```python
from build123d import *

# Parameters (mm, degrees)
CUT_EXTRUDE_1_DEPTH      = 88
CUT_EXTRUDE_1_DEPTH_BACK = 88
SKETCH_2_R               = 105
CUT_EXTRUDE_2_DEPTH      = 88
CUT_EXTRUDE_2_DEPTH_BACK = 88
SKETCH_3_R               = 5.5
CUT_EXTRUDE_3_DEPTH      = 88
CUT_EXTRUDE_3_DEPTH_BACK = 88
SKETCH_5_R               = 5.5
CUT_EXTRUDE_4_DEPTH      = 88
CUT_EXTRUDE_4_DEPTH_BACK = 88
SKETCH_6_R               = 5.5
CUT_EXTRUDE_5_DEPTH      = 88
CUT_EXTRUDE_5_DEPTH_BACK = 88
SKETCH_7_R               = 5.5
CUT_EXTRUDE_6_DEPTH      = 88
CUT_EXTRUDE_6_DEPTH_BACK = 88
SKETCH_8_R               = 5.5
CUT_EXTRUDE_7_DEPTH      = 88
CUT_EXTRUDE_7_DEPTH_BACK = 88
SKETCH_9_R               = 5.5
CUT_EXTRUDE_8_DEPTH      = 88
CUT_EXTRUDE_8_DEPTH_BACK = 88
SKETCH_10_R              = 5.5
CUT_EXTRUDE_9_DEPTH      = 88
CUT_EXTRUDE_9_DEPTH_BACK = 88
SKETCH_11_R              = 5.5


with BuildPart() as part:
    # 草图1 → 旋转1 (revolve)
    with BuildSketch(Plane.XY, mode=Mode.PRIVATE) as revolve_1_sk:
        Polygon((0, 37.5), (0, 25), (2, 23), (86, 23), (88, 25), (88, 55), (72, 55), (72, 37.5), align=None)
    revolve(revolve_1_sk.sketch.rotate(Axis((88, 0, 0), (-1, 0, 0)), 270), axis=Axis((88, 0, 0), (-1, 0, 0)))

    # 草图2 → 切除-拉伸1 (cut, two sides: drawn at the far end of the back side and taken through both)
    with BuildSketch(Plane(origin=(0, 0, 0), x_dir=(0, 0, -1), z_dir=(1, 0, 0)).offset(-CUT_EXTRUDE_1_DEPTH_BACK)):
        Circle(SKETCH_2_R)
        with BuildLine():
            Line((-42.5, 82.720916339), (-42.5, -82.720916339))
            ThreePointArc((-42.5, -82.720916339), (0, -93), (42.5, -82.720916339))
            Line((42.5, -82.720916339), (42.5, 82.720916339))
            ThreePointArc((42.5, 82.720916339), (0, 93), (-42.5, 82.720916339))
        make_face(mode=Mode.SUBTRACT)
    extrude(amount=CUT_EXTRUDE_1_DEPTH + CUT_EXTRUDE_1_DEPTH_BACK, mode=Mode.SUBTRACT)

    # 草图3 → 切除-拉伸2 (cut, two sides: drawn at the far end of the back side and taken through both)
    with BuildSketch(Plane(origin=(0, 0, 0), x_dir=(0, 0, -1), z_dir=(1, 0, 0)).offset(-CUT_EXTRUDE_2_DEPTH_BACK)):
        with Locations((-32.880465325, 32.880465325)):
            Circle(SKETCH_3_R)
    extrude(amount=CUT_EXTRUDE_2_DEPTH + CUT_EXTRUDE_2_DEPTH_BACK, mode=Mode.SUBTRACT)

    # 草图5 → 切除-拉伸3 (cut, two sides: drawn at the far end of the back side and taken through both)
    with BuildSketch(Plane(origin=(0, 0, 0), x_dir=(0, 0, -1), z_dir=(1, 0, 0)).offset(-CUT_EXTRUDE_3_DEPTH_BACK)):
        with Locations((-12.035085597, 44.915550922)):
            Circle(SKETCH_5_R)
    extrude(amount=CUT_EXTRUDE_3_DEPTH + CUT_EXTRUDE_3_DEPTH_BACK, mode=Mode.SUBTRACT)

    # 草图6 → 切除-拉伸4 (cut, two sides: drawn at the far end of the back side and taken through both)
    with BuildSketch(Plane(origin=(0, 0, 0), x_dir=(0, 0, -1), z_dir=(1, 0, 0)).offset(-CUT_EXTRUDE_4_DEPTH_BACK)):
        with Locations((12.035085597, 44.915550922)):
            Circle(SKETCH_6_R)
    extrude(amount=CUT_EXTRUDE_4_DEPTH + CUT_EXTRUDE_4_DEPTH_BACK, mode=Mode.SUBTRACT)

    # 草图7 → 切除-拉伸5 (cut, two sides: drawn at the far end of the back side and taken through both)
    with BuildSketch(Plane(origin=(0, 0, 0), x_dir=(0, 0, -1), z_dir=(1, 0, 0)).offset(-CUT_EXTRUDE_5_DEPTH_BACK)):
        with Locations((32.880465325, 32.880465325)):
            Circle(SKETCH_7_R)
    extrude(amount=CUT_EXTRUDE_5_DEPTH + CUT_EXTRUDE_5_DEPTH_BACK, mode=Mode.SUBTRACT)

    # 草图8 → 切除-拉伸6 (cut, two sides: drawn at the far end of the back side and taken through both)
    with BuildSketch(Plane(origin=(0, 0, 0), x_dir=(0, 0, -1), z_dir=(1, 0, 0)).offset(-CUT_EXTRUDE_6_DEPTH_BACK)):
        with Locations((32.880465325, -32.880465325)):
            Circle(SKETCH_8_R)
    extrude(amount=CUT_EXTRUDE_6_DEPTH + CUT_EXTRUDE_6_DEPTH_BACK, mode=Mode.SUBTRACT)

    # 草图9 → 切除-拉伸7 (cut, two sides: drawn at the far end of the back side and taken through both)
    with BuildSketch(Plane(origin=(0, 0, 0), x_dir=(0, 0, -1), z_dir=(1, 0, 0)).offset(-CUT_EXTRUDE_7_DEPTH_BACK)):
        with Locations((12.035085597, -44.915550922)):
            Circle(SKETCH_9_R)
    extrude(amount=CUT_EXTRUDE_7_DEPTH + CUT_EXTRUDE_7_DEPTH_BACK, mode=Mode.SUBTRACT)

    # 草图10 → 切除-拉伸8 (cut, two sides: drawn at the far end of the back side and taken through both)
    with BuildSketch(Plane(origin=(0, 0, 0), x_dir=(0, 0, -1), z_dir=(1, 0, 0)).offset(-CUT_EXTRUDE_8_DEPTH_BACK)):
        with Locations((-12.035085597, -44.915550922)):
            Circle(SKETCH_10_R)
    extrude(amount=CUT_EXTRUDE_8_DEPTH + CUT_EXTRUDE_8_DEPTH_BACK, mode=Mode.SUBTRACT)

    # 草图11 → 切除-拉伸9 (cut, two sides: drawn at the far end of the back side and taken through both)
    with BuildSketch(Plane(origin=(0, 0, 0), x_dir=(0, 0, -1), z_dir=(1, 0, 0)).offset(-CUT_EXTRUDE_9_DEPTH_BACK)):
        with Locations((-32.880465325, -32.880465325)):
            Circle(SKETCH_11_R)
    extrude(amount=CUT_EXTRUDE_9_DEPTH + CUT_EXTRUDE_9_DEPTH_BACK, mode=Mode.SUBTRACT)

    # 草图12 → 切除-旋转1 (revolve, cut)
    with BuildSketch(Plane(origin=(80, 0, 0), x_dir=(0, 0, -1), z_dir=(1, 0, 0)), mode=Mode.PRIVATE) as cut_revolve_1_sk:
        Polygon((7.5, 12.990381057), (4.901923789, 14.490381057), (16.901923789, 35.274990748), (16.621764571, 35.436740748), (24.283514571, 48.707281022), (24.035898385, 49.631397208), (27.5, 47.631397208), align=None)
    revolve(cut_revolve_1_sk.sketch.rotate(Axis((80, 47.631397208, -27.5), (0, -0.8660254037844387, 0.49999999999999983)), 180), axis=Axis((80, 47.631397208, -27.5), (0, -0.8660254037844387, 0.49999999999999983)), mode=Mode.SUBTRACT)


solid = part.part
```
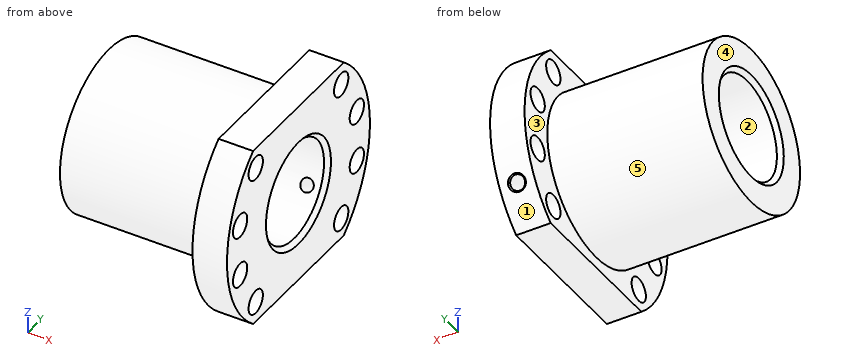
Work out the finished part from the listing and answer in its coordinate system (mm). Face numbers are marked on the shaded views. A direction names the side the tool comes from. Give positions to 0.01 mm unless a question says otherwise; leave off trailing zeros. Order: outer loops, then holes, each group sorted by start corner. A loop starts at its lowest first (then second) coordinate and runs counter-clockwise, first axis right, second up. Notation, with made-up numbers: (6.5, 54) -> (61.5, 54) arc R17 cw to (61.5, 60) -> close; hole circle Ø11 at (63, 11). An arc over 180 degrees is marked (long way). Answer as CSV lines item,"result". Start each with the question number.
(1) Consider line 1 along Z through (x, y) = (81, -32.5); line 2 along Y through (x, z) = (67.5, 0); line 3 along Y through (x, z) = (73, 35.5). Determine where each line is inside the solid, lowest interval first.
(2) For a pull along Y with two mould halves and no side action, classify the marked faces 1, 2 and 3 as released by +Y, released by -Y, zero draft, split by the parting line, or undercut.
(3) Section A-A, the plane z = 0 is taken. Write down the section's boundary in (x, y).
(4) Section B-B, the plane y = 0 is taken. Write down the section's boundary in (x, z), plus the area to 3 significant figures.
(5) Section D-D, the plane x = 53 is taken. Write down the section's boundary in (y, z).
(6) Which of the six approach directions +Z, -Z, +X, -X, +Y, -Y give full straight-line access (tool end or side, diameter ignored) to the marked faces 4 and 5?
(7) Each of these flat-tipped pins is pushed along its axis until it touches: pin 1 Ø12.5 at (y, z) = (32.88, -32.88) entering from -X; pin 2 Ø1 at (x, y) = (49, 13) entering from +Z; pin 3 Ø2 at (x, z) = (68, -30) entering from +Y (3 decimals). Where does it stop, or does it pass through?
(8) Section C-C, the plane y = -29 is taken. Write down the section's boundary in (x, z), plus the area to 3 significant figures.
Entries:
1,line 1,"-42.5 to -38.37, -27.39 to 27.39, 38.37 to 42.5"
1,line 2,"-37.5 to -23, 23 to 37.5"
1,line 3,"-42.01 to -37.72, -28.04 to 28.04, 37.72 to 42.01"
2,face 1,"released by +Y"
2,face 2,"undercut"
2,face 3,"zero draft"
3,outline,"(0, -37.5) -> (72, -37.5) -> (72, -55) -> (88, -55) -> (88, -25) -> (86, -23) -> (2, -23) -> (0, -25) -> close; (0, 25) -> (2, 23) -> (86, 23) -> (88, 25) -> (88, 55) -> (72, 55) -> (72, 37.5) -> (0, 37.5) -> close"
4,outline,"(0, -37.5) -> (72, -37.5) -> (72, -42.5) -> (88, -42.5) -> (88, -25) -> (86, -23) -> (2, -23) -> (0, -25) -> close; (0, 25) -> (2, 23) -> (86, 23) -> (88, 25) -> (88, 42.5) -> (72, 42.5) -> (72, 37.5) -> (0, 37.5) -> close"
4,area,"2,700 mm²"
5,outline,"circle Ø75 at (0, 0); hole circle Ø46 at (0, 0)"
6,face 4,"+Z, -Z, -X, +Y, -Y"
6,face 5,"-X"
7,pin 1,"x = 72"
7,pin 2,"z = 35.36"
7,pin 3,"y = 23.775"
8,outline,"(0, -23.77) -> (72, -23.77) -> (72, -28.98) -> (88, -28.98) -> (88, 28.98) -> (72, 28.98) -> (72, 23.77) -> (0, 23.77) -> close; (72, -42.5) -> (88, -42.5) -> (88, -36.78) -> (72, -36.78) -> close; (72, 36.78) -> (88, 36.78) -> (88, 42.5) -> (72, 42.5) -> close"
8,area,"4,530 mm²"
